```python
from build123d import *

# Parameters (mm, degrees)
SKETCH1_R           = 60
SKETCH1_R_2         = 50
BOSS_EXTRUDE1_DEPTH = 35
CHAMFER1_SIZE       = 3
CHAMFER2_SIZE       = 5
CHAMFER2_SIZE2      = 0.881634904


with BuildPart() as part:
    # Sketch1 → Boss-Extrude1 (new, symmetric)
    with BuildSketch(Plane.XY):
        Circle(SKETCH1_R)
        Circle(SKETCH1_R_2, mode=Mode.SUBTRACT)
    extrude(amount=BOSS_EXTRUDE1_DEPTH, both=True)

    # Chamfer1
    chamfer1_edges = [part.edges().sort_by_distance(p)[0] for p in [
        (-60, 0, 35),
        (-50, 0, -35),
        (-50, 0, 35),
    ]]
    chamfer(chamfer1_edges, length=CHAMFER1_SIZE)

    # Chamfer2
    chamfer2_edges = [part.edges().sort_by_distance(p)[0] for p in [
        (-60, 0, -35),
    ]]
    chamfer2_side = [part.faces().sort_by_distance(p)[0] for p in [
        (-60, 0, -1.5),
    ]]
    chamfer(chamfer2_edges, length=CHAMFER2_SIZE, length2=CHAMFER2_SIZE2, reference=chamfer2_side[0])


solid = part.part
```
Design review of the part built by this model. Coordinates are the model's own, in mm. Round coordinates to 2 decimals unless told otherwise and drop trailing zeros. Order: outer loops, then holes, each group sorted by start corner. A loop starts at its lowest first (then second) coordinate and runs counter-clockwise, first axis right, second up. Notation, with made-up numbers: (19.25, 81.5) - (70.25, 81.5) arc R23 ccw to (70.25, 101.5) - close; hole circle Ø8 at (19.25, 4.25). An arc over 180 degrees is marked (long way). Return JSON: item names as keys, results as strings.
Q1. The part is to be moulded in two halves that separate along Y. For faces 1 (the conical face through (-39.83, -30.54, -32.19)), 2 (the conical face through (56.43, 17.77, -34.76)), 3 (the flat face through (-22.2, 48.4, -35)), say which applies: pulls with the +Y half, pulls with the -Y half, needs draft (parallel to the pull), parting line crosses it, or undercut.
Computed values:
{"face 1": "undercut", "face 2": "parting line crosses it", "face 3": "needs draft"}
Q2. For pin 1 Ø12 at (y, z) = (30, -20.5) entering from +X; pin 2 Ø8 at (y, z) = (-14, -9) entering from +X; pin 3 Ø10 at (x, z) = (-18, -8.5) entering from -Y, all flat-tipped, find the tip position at first contact; note any pin that passes through.
Computed values:
{"pin 1": "stops at x = 54.99", "pin 2": "stops at x = 59.16", "pin 3": "stops at y = -58.57"}
Q3. Wall thickness on L1, parallel to Y at x = 0, z = 13; L2, parallel to X at y = 1, z = 5; L3, parallel to Y at x = -17, z = -29: over which ranges is each line inside the solid? List them lowest first. Write a range as [from, to].
Computed values:
{"L1": "y = [-60, -50], [50, 60]", "L2": "x = [-59.99, -49.99], [49.99, 59.99]", "L3": "y = [-57.54, -47.02], [47.02, 57.54]"}
Q4. Consider section A-A on y = 0. Write out the cut boundary in (x, z), plus the area to 3 significant figures.
Computed values:
{"outline": "(-60, -30) - (-59.12, -35) - (-53, -35) - (-50, -32) - (-50, 32) - (-53, 35) - (-57, 35) - (-60, 32) - close; (50, -32) - (53, -35) - (59.12, -35) - (60, -30) - (60, 32) - (57, 35) - (53, 35) - (50, 32) - close", "area": "1,370 mm2"}
Q5. Consider section C-C on z = -20. Write out the cut boundary in (x, y).
Computed values:
{"outline": "circle Ø120 at (0, 0); hole circle Ø100 at (0, 0)"}
